Check sheet for the drawn part. Datum: minimum x, y, z corner. Units: mm. Round coordinates to 2 decimals unless told otherwise and drop trailing zeros. Loops run counter-clockwise (first coordinate to the right, second up) from the corner with the lowest first, then second, coordinate; pieces in that order, holes last. Notation, with made-up numbers: (-33, 54) -> (-19, 54) arc R5 cw to (-19, 63) -> close; hole circle Ø2 at (-30.75, 15). An arc over 180 degrees is marked (long way). Use CSV: the item, a comma, the result in double quotes. Start each with the question number.
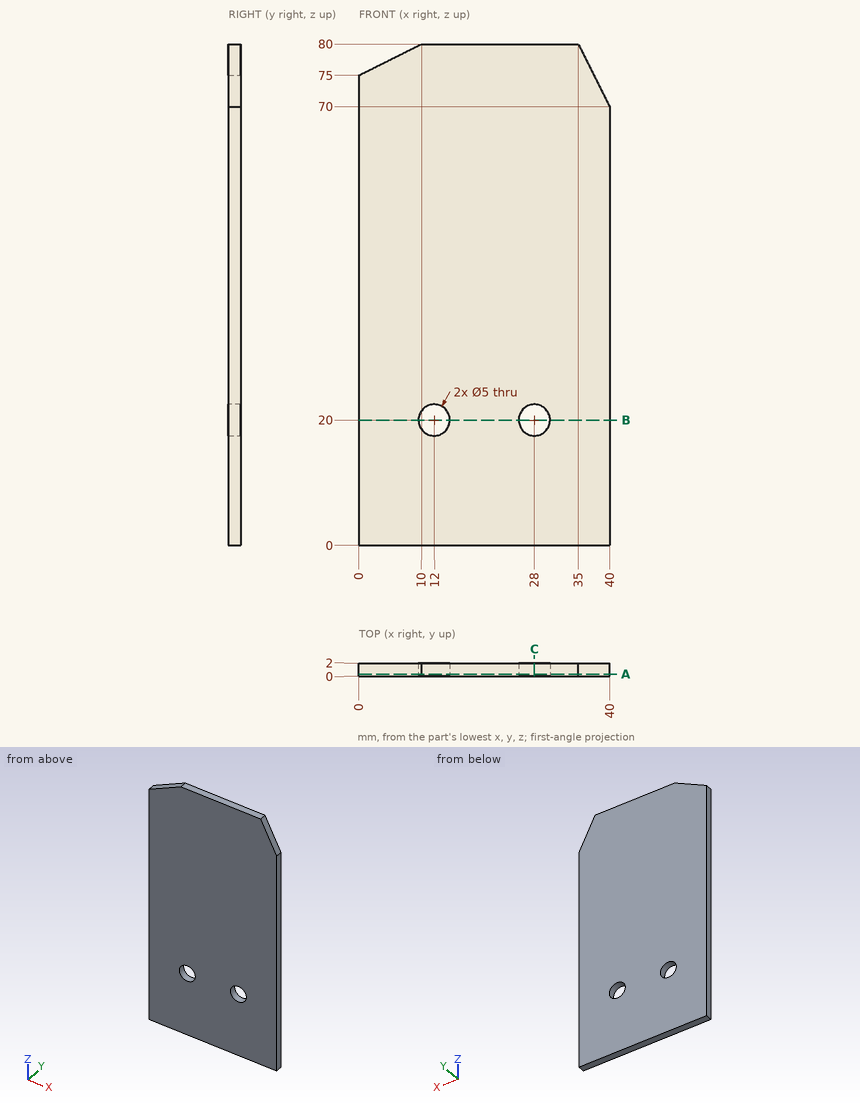
Q1. Cross-section at A-A (y = 0.3). Record the boundary of the cut face in (x, z), and give its area (3 significant figures).
Q2. Depth check by flat-ended pin: pin 1 Ø12 at (x, z) = (13, 44.5) entering from -Y; pin 2 Ø4.5 at (x, z) = (28, 20) entering from +Y. Enter the tip coordinate at first touch or a pass-through.
Q3. Cross-section at B-B (z = 20). Record the boundary of the cut face in (x, y), and give its area (3 significant figures).
Q4. Cross-section at C-C (x = 28). Record the boundary of the cut face in (y, z).
Q5. Thickness scan on L1, parallel to X at y = 1.5, z = 20; L2, parallel to X at y = 0.9, z = 22; L3, parallel to Z at x = 37, y = 0.15. Record the ranges inside material, lowest first. Write a range as from..to.
Answer list:
1,outline,"(0, 0) -> (40, 0) -> (40, 70) -> (35, 80) -> (10, 80) -> (0, 75) -> close; hole circle Ø5 at (12, 20); hole circle Ø5 at (28, 20)"
1,area,"3,110 mm2"
2,pin 1,"stops at y = 0"
2,pin 2,"passes through"
3,outline,"(0, 0) -> (9.5, 0) -> (9.5, 2) -> (0, 2) -> close; (14.5, 0) -> (25.5, 0) -> (25.5, 2) -> (14.5, 2) -> close; (30.5, 0) -> (40, 0) -> (40, 2) -> (30.5, 2) -> close"
3,area,"60.0 mm2"
4,outline,"(0, 0) -> (2, 0) -> (2, 17.5) -> (0, 17.5) -> close; (0, 22.5) -> (2, 22.5) -> (2, 80) -> (0, 80) -> close"
5,L1,"x = 0..9.5, 14.5..25.5, 30.5..40"
5,L2,"x = 0..10.5, 13.5..26.5, 29.5..40"
5,L3,"z = 0..76"
